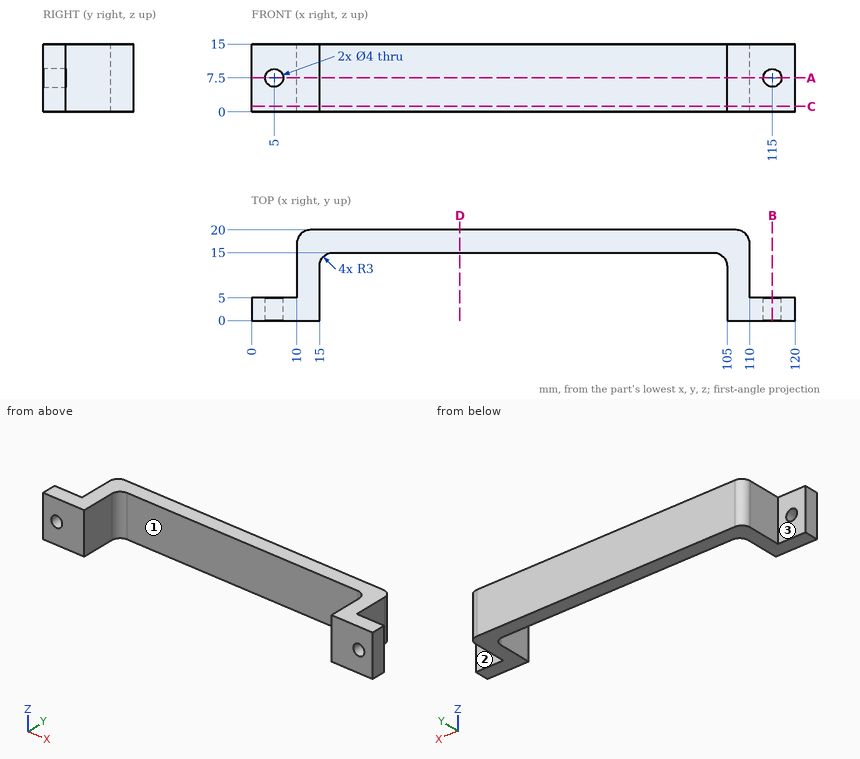
The figure shows three views and two pictorial views of one solid part (mm, origin at its lowest corner). Answer the questions. A direction names the side the tool comes from. Coordinates: 2 decimals unless noted, no trailing zeros. Loops run counter-clockwise (first coordinate to the right, second up) from the corner with the lowest first, then second, coordinate; pieces in that order, holes last. Notation, with made-up numbers: (36, 69) -> (71, 69) arc R18 cw to (71, 77) -> close; hole circle Ø11 at (-29.5, -20). An arc over 180 degrees is marked (long way). Write item = value, one per line. Start each with the question number.
1) Straight lines are drawn through the part: line 1 (X direction, y = 1.6, z = 7.5); line 2 (X direction, y = 7, z = 11.25); line 3 (X direction, y = 3.5, z = 1.5). For each, find the intervals that lie inside material, in ascending order. Write a range as from..to.
2) A cutting plane is placed at A-A (z = 7.5). Give the vertices of the cut face in (x, y).
3) A cutting plane is placed at B-B (x = 115). Give the vertices of the cut face in (y, z), then the cut area to 3 significant figures.
4) A tool of negligible diameter and unlimited length cuts with its end or side. For the marked faces 1, 2 and 3, from which of +Z, -Z, +X, -X, +Y, -Y can it reach the whole face along a straight path? Write none if from no direction.
5) A cutting plane is placed at C-C (z = 1.25). Give the vertices of the cut face in (x, y), then the cut area to 3 significant figures.
6) Given pin 1 Ø10 at (x, y) = (33.5, 12) entering from -Z; pin 2 Ø5 at (x, z) = (5, 7.5) entering from +Y; pin 3 Ø6 at (y, z) = (8.5, 3) entering from +X; pin 4 Ø3 at (y, z) = (14, 8) entering from -X, each flat-ended and moving along its own axis, determine where each tip first touches the part or whether it passes through.
7) A cutting plane is placed at D-D (x = 46). Give the vertices of the cut face in (y, z), then the cut area to 3 significant figures.
Responses:
q1.line_1 = 0..3, 7..15, 105..113, 117..120
q1.line_2 = 10..15, 105..110
q1.line_3 = 0..15, 105..120
q2.outline = (0, 0) -> (3, 0) -> (3, 5) -> (0, 5) -> close; (7, 0) -> (15, 0) -> (15, 12) arc R3 cw to (18, 15) -> (102, 15) arc R3 cw to (105, 12) -> (105, 0) -> (113, 0) -> (113, 5) -> (110, 5) -> (110, 17) arc R3 ccw to (107, 20) -> (13, 20) arc R3 ccw to (10, 17) -> (10, 5) -> (7, 5) -> close; (117, 0) -> (120, 0) -> (120, 5) -> (117, 5) -> close
q3.outline = (0, 0) -> (5, 0) -> (5, 5.5) -> (0, 5.5) -> close; (0, 9.5) -> (5, 9.5) -> (5, 15) -> (0, 15) -> close
q3.area = 55.0 mm²
q4.face_1 = +Z, -Z, -Y
q4.face_2 = +Z, -Z, +X, +Y
q4.face_3 = +Z, -Z, -X, +Y
q5.outline = (0, 0) -> (15, 0) -> (15, 12) arc R3 cw to (18, 15) -> (102, 15) arc R3 cw to (105, 12) -> (105, 0) -> (120, 0) -> (120, 5) -> (110, 5) -> (110, 17) arc R3 ccw to (107, 20) -> (13, 20) arc R3 ccw to (10, 17) -> (10, 5) -> (0, 5) -> close
q5.area = 750 mm²
q6.pin_1 = 0
q6.pin_2 = 5
q6.pin_3 = 110
q6.pin_4 = 10
q7.outline = (15, 0) -> (20, 0) -> (20, 15) -> (15, 15) -> close
q7.area = 75.0 mm²
